from build123d import *

# Parameters (mm, degrees)
SKETCH_1_R      = 5
EXTRUDE_1_DEPTH = 2


with BuildPart() as part:
    # 草图1 → 凸台-拉伸1 (new body)
    with BuildSketch(Plane(origin=(0, 0, 0), x_dir=(1, 0, 0), z_dir=(0, 1, 0))):
        with BuildLine():
            Line((0, 0), (0, 50))
            Line((0, 50), (94, 50))
            Line((94, 50), (94, -215))
            Line((94, -215), (66, -215))
            Line((66, -215), (66, -195))
            ThreePointArc((66, -195), (54, -183), (42, -195))
            Line((42, -195), (42, -215))
            Line((42, -215), (24, -215))
            Line((24, -215), (24, -170))
            Line((24, -170), (42, -152))
            Line((42, -152), (54, -152))
            ThreePointArc((54, -152), (62.485281374, -148.485281374), (66, -140))
            Line((66, -140), (66, -45))
            ThreePointArc((66, -45), (54, -33), (42, -45))
            Line((42, -45), (42, -65))
            Line((42, -65), (26, -49))
            Line((26, -49), (26, 0))
            ThreePointArc((26, 0), (14, 12), (2, 0))
            Line((2, 0), (0, 0))
        make_face()
        with Locations(Location((39, 35, 0), (0, 0, 90))):
            Circle(SKETCH_1_R, mode=Mode.SUBTRACT)
        with Locations(Location((74, 0, 0), (0, 0, 90))):
            Circle(SKETCH_1_R, mode=Mode.SUBTRACT)
    extrude(amount=EXTRUDE_1_DEPTH)


solid = part.part
The listing builds one solid part. Answer for the finished solid, in the listing's coordinates (mm). A direction names the side the tool comes from. Coordinates: 2 decimals unless noted, no trailing zeros. Write each loop counter-clockwise with the first axis right and the second up, starting at its lowest first coordinate (ties: lowest second). Pieces come first, ordered by that corner, then holes. Notation, with made-up numbers: M -20,55.5 L 37,55.5 A27 ccw 37,82.5 Z; hole C -11,-29 d4. An arc over 180 degrees is marked long. Put each result on its own line as item: value. Start each with the question number.
1. A cutting plane is placed at B-B on z = -35. Write down the section's boundary in (x, y).
2. Which of the six approach directions +Z, -Z, +X, -X, +Y, -Y give full straight-line access (tool end or side, diameter ignored) to faces 1 (the cylindrical face through (14, 1, -12)), 2 (the flat face through (33, 1, 161)), 3 (the flat face through (69, 0, 81))?
3. Consider line 1 (Z direction, x = 74, y = 0.5); line 2 (X direction, y = 1.45, z = -35); line 3 (Z direction, x = 39, y = 1.35). Determine where each line is inside the solid, lowest interval first. Write a range as from..to.
4. A cutting plane is placed at A-A on x = 74. Write down the section's boundary in (y, z).
5. A cutting plane is placed at C-C on y = 0.95. Write down the section's boundary in (x, z), then the cut area to 3 significant figures.
6. Flat-ended cylindrical pins translate along their axes: P1, Ø1, axis at y = 1.5, z = 85.5, coming from the -X side; P2, Ø1, axis at y = 0.5, z = 23, coming from the -X side; P3, Ø1, axis at y = 1, z = 207.5, coming from the -X side. Find the tip coordinate at first contact, or state that the pin passes through.
7. A cutting plane is placed at D-D on z = 173.5. Write down the section's boundary in (x, y), then the cut area to 3 significant figures.
8. For a pull along X with two mould halves and no side action, classify faces 4 (the flat face through (69, 2, 81)), 5 (the cylindrical face through (62.39, 0.99, 148.58)), 6 (the cylindrical face through (54, 1, 183)) as pulls with the +X half, pulls with the -X half, needs draft (parallel to the pull), parting line crosses it, or undercut.
Resolved:
1. outline: M 0,0 L 34,0 L 34,2 L 0,2 Z; M 44,0 L 94,0 L 94,2 L 44,2 Z
2. face 1: +Y, -Y
2. face 2: -X, +Y, -Y
2. face 3: +Z, -Z, +X, -X, -Y
3. line 1: z = -50..-5, 5..215
3. line 2: x = 0..34, 44..94
3. line 3: z = -50..-40, -30..62, 155..215
4. outline: M 0,-50 L 2,-50 L 2,-5 L 0,-5 Z; M 0,5 L 2,5 L 2,215 L 0,215 Z
5. outline: M 0,-50 L 94,-50 L 94,215 L 66,215 L 66,195 A12 cw 42,195 L 42,215 L 24,215 L 24,170 L 42,152 L 54,152 A12 cw 66,140 L 66,45 A12 cw 42,45 L 42,65 L 26,49 L 26,0 A12 cw 2,0 L 0,0 Z; hole C 39,-35 d10; hole C 74,0 d10
5. area: 13,900 mm2
6. P1: stops at x = 66
6. P2: stops at x = 26
6. P3: stops at x = 24
7. outline: M 24,0 L 94,0 L 94,2 L 24,2 Z
7. area: 140 mm2
8. face 4: needs draft
8. face 5: pulls with the -X half
8. face 6: undercut
